from build123d import *

# Parameters (mm, degrees)
SKETCH_1_R             = 10
EXTRUDE_1_DEPTH        = 500
HOLE_WIZARD_M5_1_D     = 4.2
HOLE_WIZARD_M5_1_DEPTH = 12.4
HOLE_WIZARD_M5_1_TIP   = 1.2618073
HOLE_WIZARD_M5_2_D     = 4.2
HOLE_WIZARD_M5_2_DEPTH = 12.4
HOLE_WIZARD_M5_2_TIP   = 1.2618073


with BuildPart() as part:
    # 草图1 → 凸台-拉伸1 (new body)
    with BuildSketch(Plane.XY):
        Circle(SKETCH_1_R)
    extrude(amount=EXTRUDE_1_DEPTH)

    # M5 螺纹孔1
    with Locations(Plane(origin=(0, 0, 0), x_dir=(-1, 0, 0), z_dir=(0, 0, -1))):
        with Locations((0, 0)):
            Hole(HOLE_WIZARD_M5_1_D / 2, depth=HOLE_WIZARD_M5_1_DEPTH)
            with Locations((0, 0, -(HOLE_WIZARD_M5_1_DEPTH + HOLE_WIZARD_M5_1_TIP / 2))):  # 118° drill point
                Cone(0, HOLE_WIZARD_M5_1_D / 2, HOLE_WIZARD_M5_1_TIP, mode=Mode.SUBTRACT)

    # M5 螺纹孔2
    with Locations(Plane.XY.offset(500)):
        with Locations((0, 0)):
            Hole(HOLE_WIZARD_M5_2_D / 2, depth=HOLE_WIZARD_M5_2_DEPTH)
            with Locations((0, 0, -(HOLE_WIZARD_M5_2_DEPTH + HOLE_WIZARD_M5_2_TIP / 2))):  # 118° drill point
                Cone(0, HOLE_WIZARD_M5_2_D / 2, HOLE_WIZARD_M5_2_TIP, mode=Mode.SUBTRACT)


solid = part.part
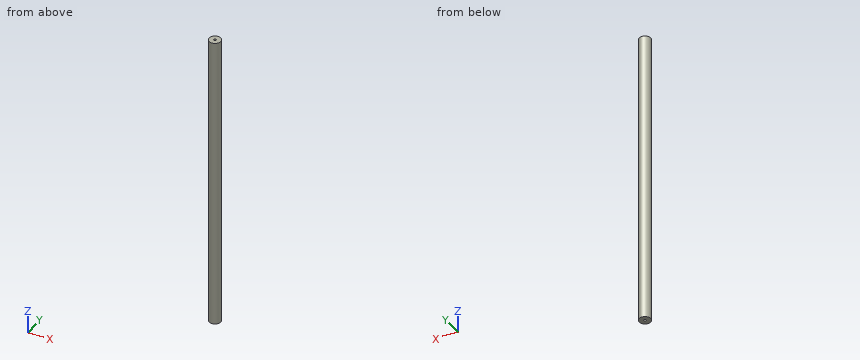
Build history of the part. All positions in model axes, mm. Give positions to 0.01 mm unless a question says otherwise; leave off trailing zeros. Order: outer loops, then holes, each group sorted by start corner. A loop starts at its lowest first (then second) coordinate and runs counter-clockwise, first axis right, second up. Notation, with made-up numbers: M 36,26 L 69,26 A22 ccw 69,52 Z; hole C 28,0 d9. An arc over 180 degrees is marked long. Use one line per item in the form item = value.
1) Probe probe 1 along Y at (x, z) = (0, 495); probe 2 along Y at (x, z) = (-2, 396.5); probe 3 along X at (y, z) = (0.25, 198). List the from-to ranges inside material, lowest first.
Calculated:
probe_1 = -10 to -2.1, 2.1 to 10
probe_2 = -9.8 to 9.8
probe_3 = -10 to 10
2) Drop flat-ended pins along their axis: pin 1 (3.5 mm diameter, centred on x = 0, y = 0, fed in from -Z); pin 2 (5 mm diameter, centred on y = 2.5, z = 346, fed in from +X); pin 3 (2.5 mm diameter, centred on x = 0, y = 0, fed in from +Z); pin 4 (1.5 mm diameter, centred on x = 3.5, z = 347, fed in from +Y). Give the stop position or say it passes through.
Calculated:
pin_1 = 12.61
pin_2 = 10
pin_3 = 487.09
pin_4 = 9.61
3) Saw through at B-B (y = 6.5). Give the cut face in (x, z), plus the area to 3 significant figures.
Calculated:
outline = M -7.6,0 L 7.6,0 L 7.6,500 L -7.6,500 Z
area = 7,600 mm2
4) Saw through at A-A (z = 378.5). Give the cut face in (x, y).
Calculated:
outline = C 0,0 d20
